Read the model definition and answer for the solid it produces. Units are mm, in the model's axes. A direction names the side the tool comes from. Give positions to 0.01 mm unless a question says otherwise; leave off trailing zeros. Loops run counter-clockwise (first coordinate to the right, second up) from the corner with the lowest first, then second, coordinate; pieces in that order, holes last. Notation, with made-up numbers: (-34.75, 41) - (21.25, 41) arc R18 ccw to (21.25, 45) - close; hole circle Ø1 at (-23, 17). An arc over 180 degrees is marked (long way). Use a Markdown table: item, result. Add a question column.
Item 1: A cutting plane is placed at B-B (x = 0). Determine the outline of the cut face in (y, z), plus the area to 3 significant figures.
Item 2: Which of the six approach directions +Z, -Z, +X, -X, +Y, -Y give full straight-line access (tool end or side, diameter ignored) to faces 1 (the face through (-18, 44, 5)), 2 (the face through (8, 15, 18)), 3 (the face through (-2.343, 105.847, 0.245))?
Item 3: A cutting plane is placed at D-D (z = 12). Determine the outline of the cut face in (x, y), plus the area to 3 significant figures.
Item 4: A cutting plane is placed at C-C (y = 96). Determine the outline of the cut face in (x, z), plus the area to 3 significant figures.
Item 5: Consider probe 1 along X at (y, z) = (4.75, -22); probe 2 along Z at (x, y) = (30, 7.5); probe 3 along Y at (x, z) = (-7.5, 13). Determine where each line is inside the solid, lowest interval first. Write a range as [from, to].
Item 6: A cutting plane is placed at A-A (z = 0.5). Determine the outline of the cut face in (x, y).
Item 7: Each of these flat-tipped pins is pushed along its axis until it touches: P1, Ø4, axis at y = 69.5, z = -15, coming from the -X side; P2, Ø13.5, axis at x = -13.5, z = 13, coming from the +Y side; P3, Ø19, axis at y = 37, z = -20, coming from the +X side. Where does it stop, or does it pass through?
Item 8: For a pull along Z with two mould halves and no side action, classify faces 4 (the face through (-40, 7, 0)), 5 (the face through (-18, 44, -5)), 6 (the face through (32.747, 6.187, 21.879)) as +Z half, -Z half, draft (parallel to the pull), parting line (faces both ways), or undercut.
from build123d import *

# Parameters (mm, degrees)
BASE_PLATE_DEPTH                        = 15
BEARING_BOSS_SKETCH_R                   = 18
BEARING_BOSS_SKETCH_R_2                 = 11.5
BEARING_BOSS_36_BORE_23_DEPTH           = 17.5
UPRIGHT_WEB_DEPTH                       = 5
MOUNTING_HOLES_M5_CSK_D                 = 5.5
MOUNTING_HOLES_M5_CSK_CSINK_D           = 10.4
MOUNTING_HOLES_M5_CSK_CSINK_ANGLE       = 90
SUPPORT_RIB_REACH                       = 119.729
SUPPORT_RIB_SKETCH_WALL_W               = 292.839761494
SUPPORT_RIB_SKETCH_WALL_H               = 10
RIB_FILLET_R7_5_R                       = 7.5
RIB_FILLET_R7_5_OF_SUPPORT_RIB_MIRROR_R = 7.5


with BuildPart() as part:
    # Base Plate Sketch → Base Plate (new body)
    with BuildSketch(Plane(origin=(0, 0, 0), x_dir=(1, 0, 0), z_dir=(0, 1, 0))):
        with BuildLine():
            Line((40, 0), (40, 22))
            ThreePointArc((40, 22), (37.071067812, 29.071067812), (30, 32))
            Line((30, 32), (-30, 32))
            ThreePointArc((-30, 32), (-37.071067812, 29.071067812), (-40, 22))
            Line((-40, 22), (-40, -22))
            ThreePointArc((-40, -22), (-37.071067812, -29.071067812), (-30, -32))
            Line((-30, -32), (30, -32))
            ThreePointArc((30, -32), (37.071067812, -29.071067812), (40, -22))
            Line((40, -22), (40, 0))
        make_face()
    extrude(amount=BASE_PLATE_DEPTH)



with BuildPart() as body_2:
    # Bearing Boss Sketch → Bearing Boss Ø36 Bore Ø23 (new, symmetric)
    with BuildSketch(Plane.XY):
        with Locations((0, 88)):
            Circle(BEARING_BOSS_SKETCH_R)
        with Locations((0, 88)):
            Circle(BEARING_BOSS_SKETCH_R_2, mode=Mode.SUBTRACT)
    extrude(amount=BEARING_BOSS_36_BORE_23_DEPTH, both=True)


with BuildPart() as part_1:
    add(part.part)

    add(body_2.part)  # Upright Web merges body 2
    # Upright Web Sketch → Upright Web (add, symmetric)
    with BuildSketch(Plane.XY):
        with BuildLine():
            Line((18, 88), (40, 15))
            Line((40, 15), (-40, 15))
            Line((-40, 15), (-18, 88))
            ThreePointArc((-18, 88), (0, 70), (18, 88))
        make_face()
    extrude(amount=UPRIGHT_WEB_DEPTH, both=True)

    # Mounting Holes M5 CSK (through all)
    with Locations(Plane(origin=(0, 15, 0), x_dir=(1, 0, 0), z_dir=(0, 1, 0))):
        with Locations((-30, 22), (30, 22), (30, -22), (-30, -22)):
            CounterSinkHole(MOUNTING_HOLES_M5_CSK_D / 2, MOUNTING_HOLES_M5_CSK_CSINK_D / 2, counter_sink_angle=MOUNTING_HOLES_M5_CSK_CSINK_ANGLE)

    # Support Rib Sketch wall → Support Rib (add, up to next)
    with BuildSketch(Plane(origin=(0, 42.5, -18.75), x_dir=(0, -0.993088841064, -0.117365044853), z_dir=(0, 0.117365044853, -0.993088841064)), mode=Mode.PRIVATE) as support_rib_sk1:
        Rectangle(SUPPORT_RIB_SKETCH_WALL_W, SUPPORT_RIB_SKETCH_WALL_H)
    support_rib_tool1 = extrude(support_rib_sk1.sketch, amount=-SUPPORT_RIB_REACH, mode=Mode.PRIVATE) - part_1.part
    support_rib = support_rib_tool1.solids().sort_by_distance((0, 42.5, -18.75))[0]
    add(support_rib)

    # Rib Fillet R7.5
    rib_fillet_r7_5_edges = [part_1.edges().sort_by_distance(p)[0] for p in [
        (0, 15, -22),
    ]]
    fillet(rib_fillet_r7_5_edges, radius=RIB_FILLET_R7_5_R)

    # Support Rib Mirror: Support Rib across plane
    add(support_rib.mirror(Plane.XY))

    # Rib Fillet R7.5 of Support Rib Mirror
    rib_fillet_r7_5_of_support_rib_mirror_edges = [part_1.edges().sort_by_distance(p)[0] for p in [
        (0, 15, 22),
    ]]
    fillet(rib_fillet_r7_5_of_support_rib_mirror_edges, radius=RIB_FILLET_R7_5_OF_SUPPORT_RIB_MIRROR_R)


solid = part_1.part
Geometry says:
| question | item | result |
|---|---|---|
| 1 | outline | (0, -32) - (15, -32) - (15, -28.67) arc R7.5 cw to (21.62, -21.22) - (70, -15.5) - (70, -17.5) - (76.5, -17.5) - (76.5, 17.5) - (70, 17.5) - (70, 15.5) - (21.62, 21.22) arc R7.5 cw to (15, 28.67) - (15, 32) - (0, 32) - close; (99.5, -17.5) - (106, -17.5) - (106, 17.5) - (99.5, 17.5) - close |
| 1 | area | 3,500 mm² |
| 2 | face 1 | +Z, -X |
| 2 | face 2 | +Z |
| 2 | face 3 | none |
| 3 | outline | (-40, 0) - (40, 0) - (40, 15) - (5, 15) - (5, 70.71) arc R18 ccw (long way) to (-5, 70.71) - (-5, 15) - (-40, 15) - close; hole circle Ø23 at (0, 88) |
| 3 | area | 2,350 mm² |
| 4 | outline | (-16.12, -17.5) - (-8.26, -17.5) - (-8.26, 17.5) - (-16.12, 17.5) - close; (8.26, -17.5) - (16.12, -17.5) - (16.12, 17.5) - (8.26, 17.5) - close |
| 4 | area | 550 mm² |
| 5 | probe 1 | [-40, -32.75], [-27.25, 27.25], [32.75, 40] |
| 5 | probe 2 | [-32, -24.75], [-19.25, 19.25], [24.75, 32] |
| 5 | probe 3 | [0, 15], [71.64, 79.28], [96.72, 104.36] |
| 6 | outline | (-40, 0) - (40, 0) - (40, 15) - (18, 88) arc R18 ccw to (-18, 88) - (-40, 15) - close; hole circle Ø23 at (0, 88) |
| 7 | P1 | x = -7.19 |
| 7 | P2 | y = 104.69 |
| 7 | P3 | x = 5 |
| 8 | face 4 | draft |
| 8 | face 5 | -Z half |
| 8 | face 6 | undercut |
